The model under review builds one solid part; all positions refer to its coordinate system, in mm. Give positions to 0.01 mm unless a question says otherwise; leave off trailing zeros. Loops run counter-clockwise (first coordinate to the right, second up) from the corner with the lowest first, then second, coordinate; pieces in that order, holes last. Notation, with made-up numbers: (5.25, 44) - (47.25, 44) arc R30 ccw to (47.25, 79) - close; hole circle Ø7 at (18, -39). An arc over 180 degrees is marked (long way). Return JSON: item names as keys, results as strings. Group by question number.
from build123d import *

# Parameters (mm, degrees)
SKETCH_1_R      = 18.25
SKETCH_1_R_2    = 8.4
SKETCH_1_R_3    = 2.25
EXTRUDE_1_DEPTH = 1
CHAMFER_1_SIZE  = 0.8


with BuildPart() as part:
    # 草图1 → 凸台-拉伸1 (new body)
    with BuildSketch(Plane.XY):
        Circle(SKETCH_1_R)
        Circle(SKETCH_1_R_2, mode=Mode.SUBTRACT)
        with Locations((0, 15)):
            Circle(SKETCH_1_R_3, mode=Mode.SUBTRACT)
        with Locations((12.990381057, -7.5)):
            Circle(SKETCH_1_R_3, mode=Mode.SUBTRACT)
        with Locations((-12.990381057, -7.5)):
            Circle(SKETCH_1_R_3, mode=Mode.SUBTRACT)
    extrude(amount=EXTRUDE_1_DEPTH)

    # 倒角1
    chamfer_1_edges = [part.edges().sort_by_distance(p)[0] for p in [
        (10.740381057, -7.5, 1),
        (-15.240381057, -7.5, 1),
        (-2.25, 15, 1),
    ]]
    chamfer(chamfer_1_edges, length=CHAMFER_1_SIZE)


solid = part.part
Item 1: For L1, parallel to Y at x = 0, z = 0.15; L2, parallel to Y at x = 0, z = 0.7; L3, parallel to Y at x = -14.5, z = 0.25, list the stretches that pass through material, from the lowest coordinate up. Write a range as from..to.
Item 2: Mouldability with a two-part tool opening along Y and no side actions: class faces 1 (the face through (-3.956, -17.816, 0.493)), 2 (the face through (8.012, 2.523, 0.493)), 3 (the face through (4, -8, 1)) as +Y half, -Y half, draft (parallel to the pull), parting line (faces both ways), or undercut.
Item 3: Take a section at D-D (z = 0.75). State the section outline as (x, y) points.
Item 4: For P1, Ø1, axis at x = -11.5, y = -7, coming from the -Z side, flat-tipped, find the tip position at first contact; note if it passes through.
Item 5: Take a section at C-C (y = 2). State the section outline as (x, z) points.
Item 6: Take a section at A-A (x = 0). State the section outline as (y, z) points.
Item 7: Take a section at B-B (y = -7.5). State the section outline as (x, z) points.
Check sheet entries:
{
 "1": {"L1": "y = -18.25..-8.4, 8.4..12.75, 17.25..18.25", "L2": "y = -18.25..-8.4, 8.4..12.25, 17.75..18.25", "L3": "y = -11.08..-9.24, -5.76..11.08"},
 "2": {"face 1": "parting line", "face 2": "undercut", "face 3": "draft"},
 "3": {"outline": "circle Ø36.5 at (0, 0); hole circle Ø5.6 at (-12.99, -7.5); hole circle Ø16.8 at (0, 0); hole circle Ø5.6 at (0, 15); hole circle Ø5.6 at (12.99, -7.5)"},
 "4": {"P1": "passes through"},
 "5": {"outline": "(-18.14, 0) - (-8.16, 0) - (-8.16, 1) - (-18.14, 1) - close; (8.16, 0) - (18.14, 0) - (18.14, 1) - (8.16, 1) - close"},
 "6": {"outline": "(-18.25, 0) - (-8.4, 0) - (-8.4, 1) - (-18.25, 1) - close; (8.4, 0) - (12.75, 0) - (12.75, 0.2) - (11.95, 1) - (8.4, 1) - close; (17.25, 0) - (18.25, 0) - (18.25, 1) - (18.05, 1) - (17.25, 0.2) - close"},
 "7": {"outline": "(-16.64, 0) - (-15.24, 0) - (-15.24, 0.2) - (-16.04, 1) - (-16.64, 1) - close; (-10.74, 0) - (-3.78, 0) - (-3.78, 1) - (-9.94, 1) - (-10.74, 0.2) - close; (3.78, 0) - (10.74, 0) - (10.74, 0.2) - (9.94, 1) - (3.78, 1) - close; (15.24, 0) - (16.64, 0) - (16.64, 1) - (16.04, 1) - (15.24, 0.2) - close"}
}
